For this review, use the dimensioned drawing (mm, ordinates from the lowest corner) and the shaded views. A direction names the side the tool comes from. Coordinates: 2 decimals unless noted, no trailing zeros. Loops run counter-clockwise (first coordinate to the right, second up) from the corner with the lowest first, then second, coordinate; pieces in that order, holes last. Notation, with made-up numbers: (44, -25.5) - (94, -25.5) arc R18 ccw to (94, -20.5) - close; hole circle Ø6 at (8, -15.75). An arc over 180 degrees is marked (long way). Answer in a Markdown table with one row per item. Add a question column.
(1) Mouldability with a two-part tool opening along X and no side actions: class the marked faces 4, 5 and 6 as +X half, -X half, draft (parallel to the pull), parting line (faces both ways), or undercut.
(2) For P1, Ø5, axis at y = 12.5, z = 8.75, coming from the -X side; P2, Ø2.5, axis at x = 5, y = 5, coming from the +Z side; P3, Ø5, axis at y = 12.5, z = 8.75, coming from the +X side, all flat-tipped, find the tip position at first contact; note any pin that passes through.
(3) For line 1 along Y through (x, z) = (5, 12.5); line 2 along Y through (x, z) = (6.75, 8.75); line 3 along Y through (x, z) = (6, 10), list the stretches that pass through material, from the lowest coordinate up.
(4) Machinability: for the marked faces 1, 2 and 3, which of the approach directions +Z, -Z, +X, -X, +Y, -Y give a long, thin tool a straight path to every point of the face, cutting with its end or side? Answer none if there is none.
(5) We need section C-C on z = 17.5. Write out the cut boundary in (x, y), plus the area to 3 significant figures.
(6) We need section B-B on z = 9.25. Write out the cut boundary in (x, y), plus the area to 3 significant figures.
(7) We need section A-A on x = 8.5. Write out the cut boundary in (y, z).
(8) We need section D-D on x = 2.5. Write out the cut boundary in (y, z), plus the area to 3 significant figures.
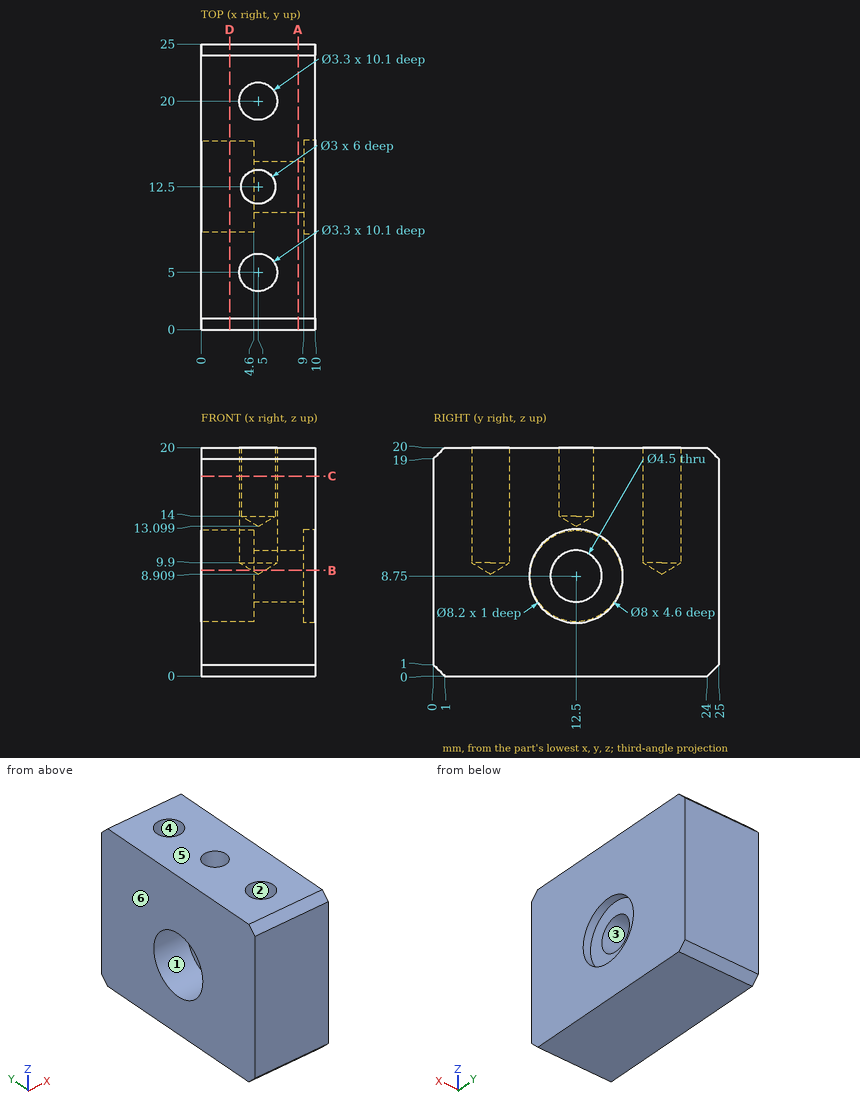
Outcome:
| question | item | result |
|---|---|---|
| 1 | face 4 | undercut |
| 1 | face 5 | draft |
| 1 | face 6 | -X half |
| 2 | P1 | x = 4.6 |
| 2 | P2 | z = 9.66 |
| 2 | P3 | x = 9 |
| 3 | line 1 | 0 to 3.35, 6.65 to 18.35, 21.65 to 25 |
| 3 | line 2 | 0 to 10.25, 14.75 to 25 |
| 3 | line 3 | 0 to 3.69, 6.31 to 10.63, 14.37 to 18.69, 21.31 to 25 |
| 4 | face 1 | -X |
| 4 | face 2 | +Z |
| 4 | face 3 | +X, -X |
| 5 | outline | (0, 0) - (10, 0) - (10, 25) - (0, 25) - close; hole circle Ø3.3 at (5, 5); hole circle Ø3.3 at (5, 20); hole circle Ø3 at (5, 12.5) |
| 5 | area | 226 mm² |
| 6 | outline | (0, 0) - (10, 0) - (10, 8.43) - (9, 8.43) - (9, 10.31) - (4.6, 10.31) - (4.6, 8.53) - (0, 8.53) - close; (0, 16.47) - (4.6, 16.47) - (4.6, 14.69) - (9, 14.69) - (9, 16.57) - (10, 16.57) - (10, 25) - (0, 25) - close; hole circle Ø1.14 at (5, 5); hole circle Ø1.14 at (5, 20) |
| 6 | area | 184 mm² |
| 7 | outline | (0, 1) - (1, 0) - (24, 0) - (25, 1) - (25, 19) - (24, 20) - (1, 20) - (0, 19) - close; hole circle Ø4.5 at (12.5, 8.75) |
| 8 | outline | (0, 1) - (1, 0) - (24, 0) - (25, 1) - (25, 19) - (24, 20) - (1, 20) - (0, 19) - close; hole circle Ø8 at (12.5, 8.75) |
| 8 | area | 448 mm² |
